Read the model definition and answer for the solid it produces. Units are mm, in the model's axes. Coordinates: 2 decimals unless noted, no trailing zeros. Order: outer loops, then holes, each group sorted by start corner. A loop starts at its lowest first (then second) coordinate and runs counter-clockwise, first axis right, second up.
```python
from build123d import *

# Parameters (mm, degrees)
SKETCH1_R           = 2.5
BOSS_EXTRUDE1_DEPTH = 4
CHAMFER1_SIZE       = 0.1


with BuildPart() as part:
    # Sketch1 → Boss-Extrude1 (new body)
    with BuildSketch(Plane(origin=(0, 0, 0), x_dir=(1, 0, 0), z_dir=(0, 1, 0))):
        Polygon((2.5, -4.330127019), (5, 0), (2.5, 4.330127019), (-2.5, 4.330127019), (-5, 0), (-2.5, -4.330127019), align=None)
        with Locations(Location((0, 0, 0), (0, 0, 270))):
            Circle(SKETCH1_R, mode=Mode.SUBTRACT)
    extrude(amount=BOSS_EXTRUDE1_DEPTH)

    # Chamfer1
    chamfer1_edges = [part.edges().sort_by_distance(p)[0] for p in [
        (0, 0, -2.5),
        (0, 4, -2.5),
    ]]
    chamfer(chamfer1_edges, length=CHAMFER1_SIZE)


solid = part.part
```
1) Determine the mould class of faces 1 (the cylindrical face through (-2.44, 1.97, -0.54)), 2 (the flat face through (2, 0, -2)), 3 (the flat face through (3.73, 1.97, 2.2)), 4 (the flat face through (0, 2, -4.33)) for opening direction Z: pulls with the +Z half, pulls with the -Z half, needs draft (parallel to the pull), parting line crosses it, or undercut.
A:
face 1: undercut
face 2: needs draft
face 3: pulls with the +Z half
face 4: pulls with the -Z half
2) A cutting plane is placed at B-B, the plane y = 2.05. Determine the outline of the cut face in (x, z).
A:
outline: (-5, 0) - (-2.5, -4.33) - (2.5, -4.33) - (5, 0) - (2.5, 4.33) - (-2.5, 4.33) - close; hole circle Ø5 at (0, 0)
3) A cutting plane is placed at A-A, the plane x = 0. Determine the outline of the cut face in (y, z), and give its area (3 significant figures).
A:
outline: (0, -4.33) - (4, -4.33) - (4, -2.6) - (3.9, -2.5) - (0.1, -2.5) - (0, -2.6) - close; (0, 2.6) - (0.1, 2.5) - (3.9, 2.5) - (4, 2.6) - (4, 4.33) - (0, 4.33) - close
area: 14.6 mm2
4) A cutting plane is placed at C-C, the plane z = -2.75. Determine the outline of the cut face in (x, y), and give its area (3 significant figures).
A:
outline: (-3.41, 0) - (3.41, 0) - (3.41, 4) - (-3.41, 4) - close
area: 27.3 mm2
5) Flat-ended cylindrical pins translate along their axes: pin 1 Ø1 at (y, z) = (2, -3) entering from +X; pin 2 Ø2 at (x, y) = (3, 3) entering from -Z. Find the tip coordinate at first contact, or state that the pin passes through.
A:
pin 1: stops at x = 3.56
pin 2: stops at z = -4.33
6) A cutting plane is placed at D-D, the plane x = -3.75. Determine the outline of the cut face in (y, z), and give its area (3 significant figures).
A:
outline: (0, -2.17) - (4, -2.17) - (4, 2.17) - (0, 2.17) - close
area: 17.3 mm2
7) Straight lines are drawn through the part: line 1 (Z direction, x = 3.5, y = 2.4); line 2 (X direction, y = 1.1, z = 1); line 3 (Z direction, x = -0.5, y = 1.5). For each, find the intervals that lie inside material, in ascending order.
A:
line 1: z = -2.6 to 2.6
line 2: x = -4.42 to -2.29, 2.29 to 4.42
line 3: z = -4.33 to -2.45, 2.45 to 4.33
